Model file for the job. Use its own axes, mm. A direction names the side the tool comes from. Give positions to 0.01 mm unless a question says otherwise; leave off trailing zeros. Order: outer loops, then holes, each group sorted by start corner. A loop starts at its lowest first (then second) coordinate and runs counter-clockwise, first axis right, second up. Notation, with made-up numbers: (70, -15.75) - (87, -15.75) arc R9 cw to (87, -2.75) - close; hole circle Ø9 at (10.5, 21.25). An arc over 180 degrees is marked (long way). Return JSON: item names as keys, results as strings. Group by question number.
from build123d import *

# Parameters (mm, degrees)
SKETCH1_R           = 40
BOSS_EXTRUDE1_DEPTH = 22
SKETCH2_R           = 42.5
BOSS_EXTRUDE2_DEPTH = 80
CUT_EXTRUDE1_START  = -28
SKETCH3_W           = 65
SKETCH3_H           = 70
CUT_EXTRUDE1_DEPTH  = 80
SKETCH4_R           = 18.25
CUT_EXTRUDE2_DEPTH  = 90
SKETCH5_R           = 18.25
CUT_EXTRUDE3_DEPTH  = 56


with BuildPart() as part:
    # Sketch1 → Boss-Extrude1 (new body)
    with BuildSketch(Plane(origin=(0, 0, 0), x_dir=(1, 0, 0), z_dir=(0, 1, 0))):
        with Locations(Location((0, 0, 0), (0, 0, 270))):
            Circle(SKETCH1_R)
    extrude(amount=BOSS_EXTRUDE1_DEPTH)

    # Sketch2 → Boss-Extrude2 (add)
    with BuildSketch(Plane(origin=(0, 22, 0), x_dir=(1, 0, 0), z_dir=(0, 1, 0))):
        with Locations(Location((0, 0, 0), (0, 0, 270))):
            Circle(SKETCH2_R)
    extrude(amount=BOSS_EXTRUDE2_DEPTH)

    # Sketch3 → Cut-Extrude1 (cut)
    with BuildSketch(Plane(origin=(0, 0, 0), x_dir=(0, 0, -1), z_dir=(1, 0, 0)).offset(CUT_EXTRUDE1_START)):
        with Locations((0, 67)):
            Rectangle(SKETCH3_W, SKETCH3_H)
    extrude(amount=-CUT_EXTRUDE1_DEPTH, mode=Mode.SUBTRACT)

    # Sketch4 → Cut-Extrude2 (cut)
    with BuildSketch(Plane.XZ):
        with Locations(Location((0, 0, 0), (0, 0, 270))):
            Circle(SKETCH4_R)
    extrude(amount=-CUT_EXTRUDE2_DEPTH, mode=Mode.SUBTRACT)

    # Sketch5 → Cut-Extrude3 (cut)
    with BuildSketch(Plane.ZY.offset(28)):
        with Locations((0, 72)):
            Circle(SKETCH5_R)
    extrude(amount=-CUT_EXTRUDE3_DEPTH, mode=Mode.SUBTRACT)


solid = part.part
(1) Slice it at A-A (z = 0). Give the cut face in (x, y), and give its area (3 significant figures).
(2) Drill centre lines: L1, parallel to Z at x = 0, y = 43; L2, parallel to Y at x = 25, z = 32; L3, parallel to X at y = 54, z = 0. Where is each one in solid material? Low to high.
(3) Slice it at B-B (x = -20.5). Give the cut face in (y, z).
(4) 3-axis set-ups, long thin cutter, end or side, ignore diameter. For faces 1 (the face through (-0.392, 90.095, -2.376)), 2 (the face through (-0.359, 84.874, -18.246)), 3 (the face through (-28, 52, 0)): which of +Z, -Z, +X, -X, +Y, -Y reach the whole face in a straight line?
(5) Slice it at D-D (x = -30.5). Give the cut face in (y, z).
(6) Pull direction Z, two halves, no side cores. Call faces 4 (the face through (-34, 32, 0)), 5 (the face through (-39.05, 10.85, -8.67)), 6 (the face through (28, 72, 0)), 7 (the face through (0, 90, 9)): released by +Z, released by -Z, zero draft, split by the parting line, or undercut.
(7) Slice it at C-C (y = 38.5). Give the cut face in (x, z).
(8) Drop flat-ended pins along their axis: pin 1 Ø2 at (x, y) = (-19.5, 13.5) entering from -Z; pin 2 Ø12 at (x, z) = (-7, -14) entering from -Y; pin 3 Ø7.5 at (x, z) = (-38.5, 3) entering from +Y; pin 4 Ø2 at (x, y) = (24.5, 68.5) entering from +Z. Give the stop position or say it passes through.
Result set:
{
 "1": {"outline": "(-42.5, 22) - (-40, 22) - (-40, 0) - (-18.25, 0) - (-18.25, 53.75) - (-28, 53.75) - (-28, 32) - (-42.5, 32) - close; (-28, 90.25) - (28, 90.25) - (28, 53.75) - (18.25, 53.75) - (18.25, 0) - (40, 0) - (40, 22) - (42.5, 22) - (42.5, 102) - (-28, 102) - close", "area": "3,540 mm²"},
 "2": {"L1": "z = -42.5 to -18.25, 18.25 to 42.5", "L2": "y = 22 to 102", "L3": "x = 28 to 42.5"},
 "3": {"outline": "(0, -34.35) - (22, -34.35) - (22, -37.23) - (102, -37.23) - (102, 37.23) - (22, 37.23) - (22, 34.35) - (0, 34.35) - close; hole circle Ø36.5 at (72, 0)"},
 "4": {"face 1": "-X", "face 2": "-Y", "face 3": "+Z, -Z, -X, +Y"},
 "5": {"outline": "(0, -25.88) - (22, -25.88) - (22, -29.6) - (32, -29.6) - (32, 29.6) - (22, 29.6) - (22, 25.88) - (0, 25.88) - close"},
 "6": {"face 4": "zero draft", "face 5": "split by the parting line", "face 6": "undercut", "face 7": "undercut"},
 "7": {"outline": "(-28, -31.97) arc R42.5 ccw (long way) to (-28, 31.97) - close; hole circle Ø36.5 at (0, 0)"},
 "8": {"pin 1": "stops at z = -35.46", "pin 2": "stops at y = 0", "pin 3": "stops at y = 32", "pin 4": "stops at z = 35.41"}
}
